Build history of the part. All positions in model axes, mm. Face numbers are marked on the shaded views. A direction names the side the tool comes from. Round coordinates to 2 decimals unless told otherwise and drop trailing zeros. Loops run counter-clockwise (first coordinate to the right, second up) from the corner with the lowest first, then second, coordinate; pieces in that order, holes last. Notation, with made-up numbers: M 36.25,31 L 45.25,31 A21 ccw 45.25,49 Z; hole C 38,58 d3. An arc over 180 degrees is marked long. One line per item, written item: value.
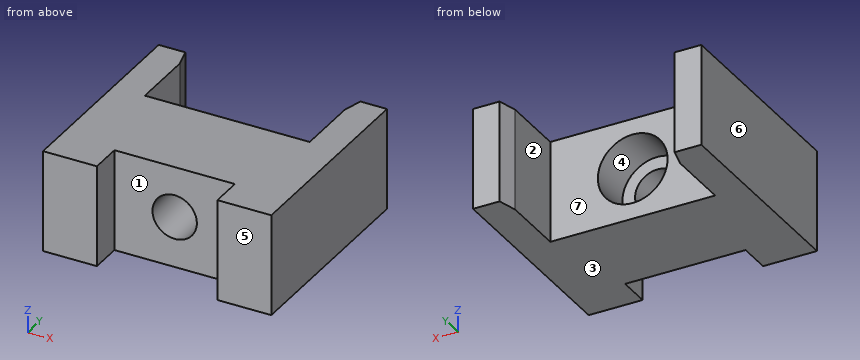
```python
from build123d import *

# Parameters (mm, degrees)
BOSS_EXTRUDE1_DEPTH = 16
SKETCH2_R           = 5.5
CUT_EXTRUDE1_DEPTH  = 7
SKETCH3_R           = 3.5
CUT_EXTRUDE2_DEPTH  = 8


with BuildPart() as part:
    # Sketch1 → Boss-Extrude1 (new body)
    with BuildSketch(Plane.XY):
        Polygon((0, 33), (0, 0), (8.5, 0), (8.5, 5), (27.5, 5), (27.5, 0), (36, 0), (36, 33), (31.803847577, 33), (31, 30), (31, 20), (5, 20), (5, 30), (4.196152423, 33), align=None)
    extrude(amount=BOSS_EXTRUDE1_DEPTH)

    # Sketch2 → Cut-Extrude1 (cut)
    with BuildSketch(Plane(origin=(0, 20, 0), x_dir=(1, 0, 0), z_dir=(0, 1, 0))):
        with Locations(Location((18, -8, 0), (0, 0, 270))):
            Circle(SKETCH2_R)
    extrude(amount=-CUT_EXTRUDE1_DEPTH, mode=Mode.SUBTRACT)

    # Sketch3 → Cut-Extrude2 (cut)
    with BuildSketch(Plane(origin=(0, 13, 0), x_dir=(1, 0, 0), z_dir=(0, 1, 0))):
        with Locations(Location((18, -8, 0), (0, 0, 270))):
            Circle(SKETCH3_R)
    extrude(amount=-CUT_EXTRUDE2_DEPTH, mode=Mode.SUBTRACT)


solid = part.part
```
Item 1: Pull direction X, two halves, no side cores. Call the marked faces 5, 6 and 7: pulls with the +X half, pulls with the -X half, needs draft (parallel to the pull), parting line crosses it, or undercut.
Check values:
face 5: needs draft
face 6: pulls with the -X half
face 7: undercut
Item 2: Which spindle directions (+Z, -Z, +X, -X, +Y, -Y) get a long thin tool onto all of the face, cutting with end or side? Do the marked faces 1, 2, 3 and 4. Say none if no direction does.
Check values:
face 1: +Z, -Z, -Y
face 2: +Z, -Z, +Y
face 3: -Z, +X, -X, +Y, -Y
face 4: +Y
Item 3: Drop flat-ended pins along their axis: P1, Ø3, axis at x = 12.5, z = 10.5, coming from the +Y side; P2, Ø6.5, axis at x = 18, z = 8, coming from the +Y side; P3, Ø12, axis at x = 13, y = 25, coming from the +Z side; P4, Ø2, axis at x = 15.5, z = 10.5, coming from the -Y side. Give the stop position or say it passes through.
Check values:
P1: stops at y = 20
P2: passes through
P3: stops at z = 16
P4: stops at y = 5
Item 4: Slice it at B-B, the plane x = 18. Give the cut face in (y, z), and give its area (3 significant figures).
Check values:
outline: M 5,0 L 20,0 L 20,2.5 L 13,2.5 L 13,4.5 L 5,4.5 Z; M 5,11.5 L 13,11.5 L 13,13.5 L 20,13.5 L 20,16 L 5,16 Z
area: 107 mm2
Item 5: Wall check: line 1 along X through (y, z) = (25, 10); line 2 along X through (y, z) = (7.25, 8); line 3 along Y through (x, z) = (14, 2.25). Give the ranges that are in metal, low to high.
Check values:
line 1: x = 0 to 5, 31 to 36
line 2: x = 0 to 14.5, 21.5 to 36
line 3: y = 5 to 20
Item 6: Slice it at C-C, the plane z = 8. Give the cut face in (x, y).
Check values:
outline: M 0,0 L 8.5,0 L 8.5,5 L 14.5,5 L 14.5,13 L 12.5,13 L 12.5,20 L 5,20 L 5,30 L 4.2,33 L 0,33 Z; M 21.5,5 L 27.5,5 L 27.5,0 L 36,0 L 36,33 L 31.8,33 L 31,30 L 31,20 L 23.5,20 L 23.5,13 L 21.5,13 Z
Item 7: Slice it at A-A, the plane y = 22. Give the cut face in (x, z), and give its area (3 significant figures).
Check values:
outline: M 0,0 L 5,0 L 5,16 L 0,16 Z; M 31,0 L 36,0 L 36,16 L 31,16 Z
area: 160 mm2
Item 8: Slice it at D-D, the plane z = 14.5. Give the cut face in (x, y), and give its area (3 significant figures).
Check values:
outline: M 0,0 L 8.5,0 L 8.5,5 L 27.5,5 L 27.5,0 L 36,0 L 36,33 L 31.8,33 L 31,30 L 31,20 L 5,20 L 5,30 L 4.2,33 L 0,33 Z
area: 753 mm2
